Work out the finished part from the listing and answer in its coordinate system (mm). A direction names the side the tool comes from. Round coordinates to 2 decimals unless told otherwise and drop trailing zeros. Loops run counter-clockwise (first coordinate to the right, second up) from the corner with the lowest first, then second, coordinate; pieces in that order, holes last. Notation, with made-up numbers: (51.25, -7.75) - (59.25, -7.75) arc R32 ccw to (59.25, 24.25) - close; hole circle Ø8 at (65, 35). An arc over 180 degrees is marked (long way). Answer as CSV lines item,"result". Start each with the question number.
```python
from build123d import *

# Parameters (mm, degrees)
EXTRUDE1_DEPTH        = 34.9
SKETCH2_R             = 4
EXTRUDE2_DEPTH        = 12
M5_TAPPED_HOLE1_D     = 4.2
M5_TAPPED_HOLE1_DEPTH = 12.4
M5_TAPPED_HOLE1_TIP   = 1.2618073


with BuildPart() as part:
    # Sketch1 → Extrude1 (new, symmetric)
    with BuildSketch(Plane.XY):
        with BuildLine():
            Line((32, -25), (44, -25))
            Line((44, -25), (44, 0))
            Line((44, 0), (0, 0))
            Line((0, 0), (0, -25))
            Line((0, -25), (12, -25))
            Line((12, -25), (12, -21.5))
            ThreePointArc((12, -21.5), (14.5, -19), (12, -16.5))
            Line((12, -16.5), (12, -12))
            Line((12, -12), (32, -12))
            Line((32, -12), (32, -16.5))
            ThreePointArc((32, -16.5), (29.5, -19), (32, -21.5))
            Line((32, -21.5), (32, -25))
        make_face()
    extrude(amount=EXTRUDE1_DEPTH, both=True)

    # Sketch2 → Extrude2 (add)
    with BuildSketch(Plane.XY.offset(34.9)):
        with Locations((22, -5)):
            Circle(SKETCH2_R)
    extrude(amount=EXTRUDE2_DEPTH)

    # M5 Tapped Hole1
    with Locations(Plane(origin=(6, 0, 18), x_dir=(0, 0, 1), z_dir=(0, 1, 0))):
        with Locations((0, 0), (0, 32), (-36, 0), (-36, 32)):
            Hole(M5_TAPPED_HOLE1_D / 2, depth=M5_TAPPED_HOLE1_DEPTH)
            with Locations((0, 0, -(M5_TAPPED_HOLE1_DEPTH + M5_TAPPED_HOLE1_TIP / 2))):  # 118° drill point
                Cone(0, M5_TAPPED_HOLE1_D / 2, M5_TAPPED_HOLE1_TIP, mode=Mode.SUBTRACT)


solid = part.part
```
Item 1: Section C-C, the plane y = -8 is taken. Give the vertices of the cut face in (x, z), and give its area (3 significant figures).
Item 2: Find the intervals of material crossed by L1, parallel to Z at x = 38, y = -9.25; L2, parallel to X at y = -9.5, z = 18; L3, parallel to X at y = -21.75, z = 29.5, in increasing order.
Item 3: Section A-A, the plane y = -23.25 is taken. Give the vertices of the cut face in (x, z), and give its area (3 significant figures).
Item 4: Which of the six approach directions +Z, -Z, +X, -X, +Y, -Y give full straight-line access (tool end or side, diameter ignored) to faces 4 (the face through (22, 0, 0)), 5 (the face through (14.5, -19.1, 0.5)), 6 (the face through (32, -23, 0)), 7 (the face through (6.631, -6.287, 15.997))?
Item 5: Section D-D, the plane y = -19 is taken. Give the vertices of the cut face in (x, z), and give its area (3 significant figures).
Item 6: Flat-ended cylindrical pins translate along their axes: pin 1 Ø1.5 at (x, z) = (22.5, 33) entering from -Y; pin 2 Ø10 at (x, y) = (28.5, -13) entering from +Z; pin 3 Ø3.5 at (x, z) = (38, -18) entering from +Y. Find the tip coordinate at first contact, or state that the pin passes through.
Item 7: Section B-B, the plane z = -7 is taken. Give the vertices of the cut face in (x, y), and give its area (3 significant figures).
Item 8: Determine the mould class of faces 1 (the face through (22, -10, -34.9)), 2 (the face through (38.25, -13.44, -18.27)), 3 (the face through (29.5, -18.9, 0.5)) for opening direction Z: pulls with the +Z half, pulls with the -Z half, needs draft (parallel to the pull), parting line crosses it, or undercut.
Answer:
1,outline,"(0, -34.9) - (44, -34.9) - (44, 34.9) - (24.65, 34.9) - (24.65, 46.9) - (19.35, 46.9) - (19.35, 34.9) - (0, 34.9) - close; hole circle Ø4.2 at (6, -18); hole circle Ø4.2 at (6, 18); hole circle Ø4.2 at (38, -18); hole circle Ø4.2 at (38, 18)"
1,area,"3,080 mm²"
2,L1,"z = -34.9 to -20.1, -15.9 to 15.9, 20.1 to 34.9"
2,L2,"x = 0 to 3.9, 8.1 to 35.9, 40.1 to 44"
2,L3,"x = 0 to 12, 32 to 44"
3,outline,"(0, -34.9) - (12, -34.9) - (12, 34.9) - (0, 34.9) - close; (32, -34.9) - (44, -34.9) - (44, 34.9) - (32, 34.9) - close"
3,area,"1,680 mm²"
4,face 4,"+Z, -Z, +X, -X, +Y"
4,face 5,"+Z, -Z"
4,face 6,"+Z, -Z, -Y"
4,face 7,"+Y"
5,outline,"(0, -34.9) - (14.5, -34.9) - (14.5, 34.9) - (0, 34.9) - close; (29.5, -34.9) - (44, -34.9) - (44, 34.9) - (29.5, 34.9) - close"
5,area,"2,020 mm²"
6,pin 1,"stops at y = -12"
6,pin 2,"stops at z = 34.9"
6,pin 3,"stops at y = -12.61"
7,outline,"(0, -25) - (12, -25) - (12, -21.5) arc R2.5 ccw to (12, -16.5) - (12, -12) - (32, -12) - (32, -16.5) arc R2.5 ccw to (32, -21.5) - (32, -25) - (44, -25) - (44, 0) - (0, 0) - close"
7,area,"860 mm²"
8,face 1,"pulls with the -Z half"
8,face 2,"undercut"
8,face 3,"needs draft"
